Input: part model. Units: mm. Frame: model coordinates. Give positions to 0.01 mm unless a question says otherwise; leave off trailing zeros. Loops run counter-clockwise (first coordinate to the right, second up) from the corner with the lowest first, then second, coordinate; pieces in that order, holes last. Notation, with made-up numbers: (3.25, 15) - (56.25, 15) arc R37 ccw to (56.25, 52) - close; hole circle Ø2 at (68, 73.25). An arc over 180 degrees is marked (long way). Answer as a JSON object with one key per item and string values.
from build123d import *

# Parameters (mm, degrees)
SKETCH1_W            = 82
SKETCH1_H            = 50
BOSS_EXTRUDE1_DEPTH  = 16
M4_TAPPED_HOLE1_D    = 3.3
LPATTERN1_COUNT      = 2
LPATTERN1_PITCH      = 38
LPATTERN1_COUNT_DIR2 = 2
LPATTERN1_PITCH_DIR2 = 25
CHAMFER1_SIZE        = 1.5


with BuildPart() as part:
    # Sketch1 → Boss-Extrude1 (new body)
    with BuildSketch(Plane.XY):
        Rectangle(SKETCH1_W, SKETCH1_H)
    extrude(amount=BOSS_EXTRUDE1_DEPTH)

    # M4 Tapped Hole1 (through all)
    with Locations(Plane(origin=(19, 12.5, 0), x_dir=(-1, 0, 0), z_dir=(0, 0, -1))):
        with Locations((0, 0)):
            m4_tapped_hole1 = Hole(M4_TAPPED_HOLE1_D / 2)

    # LPattern1: M4 Tapped Hole1 2 × 2
    with Locations(*[(-i * LPATTERN1_PITCH, -j * LPATTERN1_PITCH_DIR2, 0) for i in range(LPATTERN1_COUNT) for j in range(LPATTERN1_COUNT_DIR2) if (i, j) != (0, 0)]):
        add(m4_tapped_hole1, mode=Mode.SUBTRACT)

    # Chamfer1
    chamfer1_edges = [part.edges().sort_by_distance(p)[0] for p in [
        (0, 25, 0),
        (41, 0, 0),
        (0, -25, 0),
        (-41, 0, 0),
    ]]
    chamfer(chamfer1_edges, length=CHAMFER1_SIZE)


solid = part.part
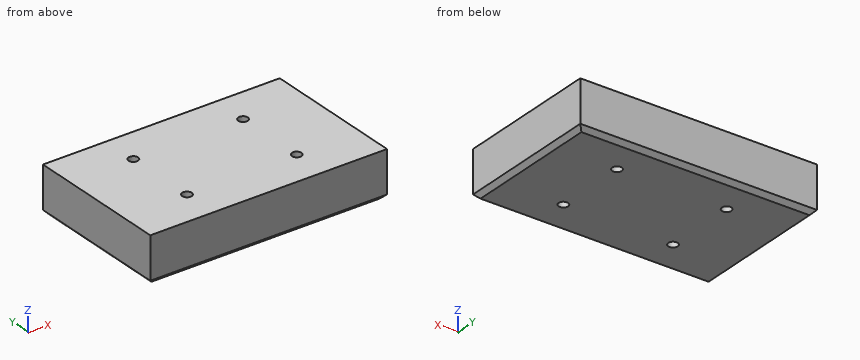
Item 1: Cut plane B-B (y = -12.5). Return loops of the section in (x, z), then the cut area to 3 significant figures.
Geometry check:
{"outline": "(-41, 1.5) - (-39.5, 0) - (-20.65, 0) - (-20.65, 16) - (-41, 16) - close; (-17.35, 0) - (17.35, 0) - (17.35, 16) - (-17.35, 16) - close; (20.65, 0) - (39.5, 0) - (41, 1.5) - (41, 16) - (20.65, 16) - close", "area": "1,200 mm2"}
Item 2: Material intervals for line 1 (Y direction, x = -19, z = 6.5); line 2 (Y direction, x = -18, z = 3.25), sorted ascending. Write a range as [from, to].
Geometry check:
{"line 1": "y = [-25, -14.15], [-10.85, 10.85], [14.15, 25]", "line 2": "y = [-25, -13.81], [-11.19, 11.19], [13.81, 25]"}
Item 3: Cut plane A-A (x = 19). Return loops of the section in (y, z), then the cut area to 3 significant figures.
Geometry check:
{"outline": "(-25, 1.5) - (-23.5, 0) - (-14.15, 0) - (-14.15, 16) - (-25, 16) - close; (-10.85, 0) - (10.85, 0) - (10.85, 16) - (-10.85, 16) - close; (14.15, 0) - (23.5, 0) - (25, 1.5) - (25, 16) - (14.15, 16) - close", "area": "692 mm2"}
